For this review, take the finished solid that the model builds, in its own axes (mm). A direction names the side the tool comes from. Coordinates: 2 decimals unless noted, no trailing zeros. Write each loop counter-clockwise with the first axis right and the second up, starting at its lowest first coordinate (ties: lowest second). Pieces come first, ordered by that corner, then holes. Notation, with made-up numbers: M -7.75,13.5 L 29.25,13.5 A27 ccw 29.25,49.5 Z; hole C 71.5,19.25 d4. An arc over 180 degrees is marked long. Return JSON: item names as keys, results as strings.
```python
from build123d import *

# Parameters (mm, degrees)
BOSS_EXTRUDE1_DEPTH   = 30
SKETCH2_W             = 120
SKETCH2_H             = 120
CUT_EXTRUDE1_DEPTH    = 30
SKETCH3_W             = 90
SKETCH3_H             = 50
CUT_EXTRUDE2_DEPTH    = 7
SHELL1_T              = -5
M4_TAPPED_HOLE1_D     = 3.3
M4_TAPPED_HOLE1_DEPTH = 10.1
M4_TAPPED_HOLE1_TIP   = 0.991420021


with BuildPart() as part:
    # Sketch1 → Boss-Extrude1 (new body)
    with BuildSketch(Plane.XY):
        Polygon((-500, 500), (0, 0), (-500, -500), align=None)
    extrude(amount=BOSS_EXTRUDE1_DEPTH)

    # Sketch2 → Cut-Extrude1 (cut)
    with BuildSketch(Plane.XY.offset(30)):
        Rectangle(SKETCH2_W, SKETCH2_H)
    extrude(amount=-CUT_EXTRUDE1_DEPTH, mode=Mode.SUBTRACT)

    # Sketch3 → Cut-Extrude2 (cut)
    with BuildSketch(Plane.ZY.offset(500)):
        with Locations((-20, 325)):
            Rectangle(SKETCH3_W, SKETCH3_H)
        with Locations((-20, -325)):
            Rectangle(SKETCH3_W, SKETCH3_H)
    extrude(amount=-CUT_EXTRUDE2_DEPTH, mode=Mode.SUBTRACT)

    # Shell1
    shell1_openings = [part.faces().sort_by_distance(p)[0] for p in [
        (-60, 0, 15),
    ]]
    offset(amount=SHELL1_T, openings=shell1_openings, kind=Kind.INTERSECTION)

    # M4 Tapped Hole1
    with Locations(Plane.ZY.offset(493)):
        with Locations((17.5, 335), (17.5, 315), (17.5, -315), (17.5, -335)):
            Hole(M4_TAPPED_HOLE1_D / 2, depth=M4_TAPPED_HOLE1_DEPTH)
            with Locations((0, 0, -(M4_TAPPED_HOLE1_DEPTH + M4_TAPPED_HOLE1_TIP / 2))):  # 118° drill point
                Cone(0, M4_TAPPED_HOLE1_D / 2, M4_TAPPED_HOLE1_TIP, mode=Mode.SUBTRACT)


solid = part.part
```
1. Draft analysis for pull direction Y (two halves, no side actions). For faces 4 (the face through (-326, 7, 0)), 5 (the face through (-493, -325, 12)), 6 (the face through (-277, -277, 15)), state which applies: +Y half, -Y half, draft (parallel to the pull), parting line (faces both ways), or undercut.
Checks:
{"face 4": "draft", "face 5": "undercut", "face 6": "-Y half"}
2. We need section B-B (x = -87). State the section outline as (y, z) points, plus the area to 3 significant figures.
Checks:
{"outline": "M -87,0 L 87,0 L 87,30 L -87,30 Z; hole M -79.93,5 L 79.93,5 L 79.93,25 L -79.93,25 Z", "area": "2,020 mm2"}
3. We need section C-C (y = 21.5). State the section outline as (x, z) points, plus the area to 3 significant figures.
Checks:
{"outline": "M -500,0 L -60,0 L -60,5 L -495,5 L -495,25 L -60,25 L -60,30 L -500,30 Z", "area": "4,500 mm2"}
4. For faces 1 (the face through (-493, 325, 12)), 2 (the face through (-500, -7, 15)), 3 (the face through (-323, 7, 25)), list the 3-axis set-ups (+Z, -Z, +X, -X, +Y, -Y) from which the entire face can be reached by the end or side of a thin tool; tool diameter is ignored.
Checks:
{"face 1": "-Z, -X", "face 2": "+Z, -Z, -X, +Y, -Y", "face 3": "none"}
5. Wall thickness on L1, parallel to Z at x = -489.95, y = -335; L2, parallel to Z at x = -384.5, y = -376; L3, parallel to Y at x = -218.5, z = 10.5: over which ranges is each line inside the solid? List them lowest first. Write a range as from..to.
Checks:
{"L1": "0..15.85, 19.15..30", "L2": "0..5, 25..30", "L3": "-218.5..-211.43, 211.43..218.5"}
6. Clearance check with flat-ended pins moving along their axes: pin 1 Ø7.5 at (x, z) = (-498, 10) entering from +Y; pin 2 Ø5 at (y, z) = (66.5, 22) entering from +X; pin 3 Ø3.5 at (x, z) = (-491.5, 18) entering from +Y; pin 4 Ø4 at (y, z) = (315, 17.5) entering from -X. State where each tip first meets the part, or that it passes through.
Checks:
{"pin 1": "y = 500", "pin 2": "x = -64", "pin 3": "y = 493.25", "pin 4": "x = -493"}
7. We need section A-A (y = 239). State the section outline as (x, z) points.
Checks:
{"outline": "M -500,0 L -239,0 L -239,30 L -500,30 Z; hole M -495,5 L -246.07,5 L -246.07,25 L -495,25 Z"}
